Input: part model. Units: mm. Frame: model coordinates. A direction names the side the tool comes from. Coordinates: 2 decimals unless noted, no trailing zeros. Write each loop counter-clockwise with the first axis right and the second up, starting at its lowest first coordinate (ties: lowest second). Pieces come first, ordered by that corner, then holes.
1) Section query A-A (x = 73.5). Output: boundary loops of the cut face in (y, z), then the cut area to 3 significant figures.
2) Section query B-B (z = 35). Output: boundary loops of the cut face in (x, y).
3) Pin query (flat end, axial travel): pin 1 Ø6 at (x, y) = (65, 24) entering from +Z; pin 2 Ø8 at (x, z) = (22.5, 41.5) entering from +Y; pin 3 Ø6.5 at (y, z) = (74.5, 4.5) entering from -X. Return the tip coordinate at first contact, or that it passes through.
4) Set-up query: faces 1 (the flat face through (20, 93, 4)), 2 (the flat face through (64.7, 8, 33.6)), 3 (the flat face through (70, 92, 4)), 4 (the flat face through (44, 72, 8)). Return all of +Z, -Z, +X, -X, +Y, -Y with unobstructed straight access to the full face (end or side cutting, diameter ignored); none if empty.
5) Line query: L1, parallel to Z at x = 70, y = 5; L2, parallel to Y at x = 73, z = 14.5; L3, parallel to X at y = 12.5, z = 45.5. Output: solid intervals per line, ascending.
6) Section query D-D (z = 6). Output: boundary loops of the cut face in (x, y), then the cut area to 3 significant figures.
7) Section query C-C (y = 17). Output: boundary loops of the cut face in (x, z), then the cut area to 3 significant figures.
from build123d import *
from build123d.topology import SkipClean

# Parameters (mm, degrees)
EXTRUDE_2_DEPTH      = 8
SKETCH_2_W           = 90
SKETCH_2_H           = 8
EXTRUDE_3_DEPTH      = 52
EXTRUDE_4_DEPTH      = 4
EXTRUDE_4_DEPTH_BACK = 4
CUT_EXTRUDE_2_DEPTH  = 18
SKETCH_6_R           = 5
CUT_EXTRUDE_3_DEPTH  = 10
SKETCH_8_R           = 5
CUT_EXTRUDE_4_DEPTH  = 10
EXTRUDE_6_DEPTH      = 8


with BuildPart() as part:
    # Sketch 1 → Extrude 2 (new body)
    with BuildSketch(Plane.XY):
        Polygon((0, 0), (90, 0), (90, 30), (70, 50), (70, 135), (45, 135), (20, 135), (20, 50), (0, 30), align=None)
    extrude(amount=EXTRUDE_2_DEPTH)

    # Sketch 2 → Extrude 3 (add)
    with BuildSketch(Plane.XY.offset(8)):
        with Locations((45, 4)):
            Rectangle(SKETCH_2_W, SKETCH_2_H)
    extrude(amount=EXTRUDE_3_DEPTH)

    # Sketch 4 → Extrude 4 (add, two sides: drawn at the far end of the back side and taken through both)
    with BuildSketch(Plane(origin=(45, 0, 0), x_dir=(0, 0, -1), z_dir=(1, 0, 0)).offset(-EXTRUDE_4_DEPTH_BACK)):
        Polygon((-8, 8), (-8, 50), (-60, 8), align=None)
    extrude(amount=EXTRUDE_4_DEPTH + EXTRUDE_4_DEPTH_BACK)

    # Sketch 5 → Cut-Extrude 2 (cut)
    with BuildSketch(Plane(origin=(0, 8, 0), x_dir=(1, 0, 0), z_dir=(0, 1, 0))):
        with BuildLine():
            ThreePointArc((70, -35), (65, -30), (60, -35))
            Line((60, -35), (65, -35))
            Line((65, -35), (70, -35))
        make_face()
        with BuildLine():
            Line((65, -35), (60, -35))
            ThreePointArc((60, -35), (65, -40), (70, -35))
            Line((70, -35), (65, -35))
        make_face()
        with BuildLine():
            Line((20, -35), (25, -35))
            Line((25, -35), (30, -35))
            ThreePointArc((30, -35), (25, -30), (20, -35))
        make_face()
        with BuildLine():
            Line((30, -35), (25, -35))
            Line((25, -35), (20, -35))
            ThreePointArc((20, -35), (25, -40), (30, -35))
        make_face()
    extrude(amount=-CUT_EXTRUDE_2_DEPTH, mode=Mode.SUBTRACT)

    # Sketch 6 → Cut-Extrude 3 (cut)
    with BuildSketch(Plane(origin=(0, 8, 0), x_dir=(1, 0, 0), z_dir=(0, 1, 0))):
        with Locations((20, -35)):
            Circle(SKETCH_6_R)
    extrude(amount=-CUT_EXTRUDE_3_DEPTH, mode=Mode.SUBTRACT)

    # Sketch 8 → Cut-Extrude 4 (cut)
    with BuildSketch(Plane(origin=(0, 8, 0), x_dir=(1, 0, 0), z_dir=(0, 1, 0))):
        with Locations((70, -35)):
            Circle(SKETCH_8_R)
        with Locations((65, -35)):
            Circle(SKETCH_8_R)
    extrude(amount=-CUT_EXTRUDE_4_DEPTH, mode=Mode.SUBTRACT)

    # Sketch 9 → Extrude 6 (add)
    with SkipClean():  # the faces are left unmerged after this step: merging them gives an invalid solid
        with BuildSketch(Plane(origin=(0, 8, 0), x_dir=(1, 0, 0), z_dir=(0, 1, 0))):
            with BuildLine():
                ThreePointArc((22.5, -30.669872981), (25, -35), (22.5, -39.330127019))
                ThreePointArc((22.5, -39.330127019), (30, -35), (22.5, -30.669872981))
            make_face()
            with BuildLine():
                ThreePointArc((67.5, -39.330127019), (65, -35), (67.5, -30.669872981))
                ThreePointArc((67.5, -30.669872981), (60, -35), (67.5, -39.330127019))
            make_face()
        extrude(amount=-EXTRUDE_6_DEPTH)


solid = part.part
Answer:
1. outline: (0, 0) - (46.5, 0) - (46.5, 8) - (8, 8) - (8, 31.43) - (0, 31.43) - close; (0, 38.57) - (8, 38.57) - (8, 60) - (0, 60) - close
1. area: 731 mm2
2. outline: (0, 0) - (15, 0) - (15, 8) - (0, 8) - close; (25, 0) - (65, 0) - (65, 8) - (49, 8) - (49, 28.19) - (41, 28.19) - (41, 8) - (25, 8) - close; (75, 0) - (90, 0) - (90, 8) - (75, 8) - close
3. pin 1: stops at z = 8
3. pin 2: stops at y = 8
3. pin 3: stops at x = 20
4. face 1: +Z, -Z, -X, +Y
4. face 2: +Z, +X, +Y
4. face 3: +Z, -Z, +X, +Y
4. face 4: +Z, +Y
5. L1: z = 0 to 30, 40 to 60
5. L2: y = 0 to 8
5. L3: x = 41 to 49
6. outline: (0, 0) - (90, 0) - (90, 30) - (70, 50) - (70, 135) - (20, 135) - (20, 50) - (0, 30) - close
6. area: 8,350 mm2
7. outline: (0, 0) - (90, 0) - (90, 8) - (49, 8) - (49, 48.86) - (41, 48.86) - (41, 8) - (0, 8) - close
7. area: 1,050 mm2
